```python
from build123d import *

# Parameters (mm, degrees)
SKETCH1_R           = 9
BOSS_EXTRUDE1_DEPTH = 4
SKETCH2_R           = 6
BOSS_EXTRUDE2_DEPTH = 2
SKETCH3_R           = 6.5
BOSS_EXTRUDE3_DEPTH = 54.2
SKETCH4_R           = 5.95
BOSS_EXTRUDE4_DEPTH = 1
SKETCH5_R           = 6.5
BOSS_EXTRUDE5_DEPTH = 4.8
CHAMFER1_SIZE       = 1


with BuildPart() as part:
    # Sketch1 → Boss-Extrude1 (new body)
    with BuildSketch(Plane.XY):
        Circle(SKETCH1_R)
    extrude(amount=BOSS_EXTRUDE1_DEPTH)

    # Sketch2 → Boss-Extrude2 (add)
    with BuildSketch(Plane.XY.offset(4)):
        Circle(SKETCH2_R)
    extrude(amount=BOSS_EXTRUDE2_DEPTH)

    # Sketch3 → Boss-Extrude3 (add)
    with BuildSketch(Plane.XY.offset(6)):
        with Locations(Location((0, 0, 0), (0, 0, 180))):
            Circle(SKETCH3_R)
    extrude(amount=BOSS_EXTRUDE3_DEPTH)

    # Sketch4 → Boss-Extrude4 (add)
    with BuildSketch(Plane.XY.offset(60.2)):
        Circle(SKETCH4_R)
    extrude(amount=BOSS_EXTRUDE4_DEPTH)

    # Sketch5 → Boss-Extrude5 (add)
    with BuildSketch(Plane.XY.offset(61.2)):
        with Locations(Location((0, 0, 0), (0, 0, 180))):
            Circle(SKETCH5_R)
    extrude(amount=BOSS_EXTRUDE5_DEPTH)

    # Chamfer1
    chamfer1_edges = [part.edges().sort_by_distance(p)[0] for p in [
        (-9, 0, 0),
        (6.5, 0, 66),
    ]]
    chamfer(chamfer1_edges, length=CHAMFER1_SIZE)


solid = part.part
```
Geometry: final body of the model. Coordinates: model frame, mm. A direction names the side the tool comes from. Round coordinates to 2 decimals unless told otherwise and drop trailing zeros. Write each loop counter-clockwise with the first axis right and the second up, starting at its lowest first coordinate (ties: lowest second). Pieces come first, ordered by that corner, then holes. Notation, with made-up numbers: (-40, -4) -> (3, -4) arc R13 ccw to (3, 12) -> close; hole circle Ø5 at (54, 3.5). An arc over 180 degrees is marked (long way). Use CSV: the item, a comma, the result in double quotes. Start each with the question number.
Q1. Reachability of faces 4 (the face through (0, 0, 0)), 5 (the face through (5.158, 3.955, 32.721)), 6 (the face through (-6, 0, 5)) from +Z, -Z, +X, -X, +Y, -Y: full face, straight path, thin tool, end or side. Return the list, or none.
Q2. First-contact query: pin 1 Ø6.5 at (x, y) = (-0.5, 2.5) entering from -Z; pin 2 Ø4 at (x, z) = (-0.5, 59) entering from +Y; pin 3 Ø8 at (y, z) = (-5, 13.5) entering from +X; pin 4 Ø10 at (y, z) = (0, 35.5) entering from +X. Flat tips, straight axial feed; report the tip coordinate or a pass-through.
Q3. Line query: L1, parallel to Z at x = 6.25, y = 1.25; L2, parallel to Z at x = 2, y = -7.25; L3, parallel to Y at x = 2.5, z = 53.5. Output: solid intervals per line, ascending.
Q4. Section A-A (x = 0). Return loops of the section in (y, z), plus the area to 3 significant figures.
Q5. Pull-direction query (Z, two-part tool) for faces 1 (the face through (0, 0, 66)), 2 (the face through (-1.172, 8.923, 2.479)), 3 (the face through (-6, 2, 61.2)); classes: pulls with the +Z half, pulls with the -Z half, needs draft (parallel to the pull), parting line crosses it, or undercut.
Q6. Section C-C (z = 59). Return loops of the section in (x, y).
Result sheet:
1,face 4,"-Z, +X, -X, +Y, -Y"
1,face 5,"+Z"
1,face 6,"none"
2,pin 1,"z = 0"
2,pin 2,"y = 6.5"
2,pin 3,"x = 6.42"
2,pin 4,"x = 6.5"
3,L1,"0 to 4, 6 to 60.2, 61.2 to 65.13"
3,L2,"0 to 4"
3,L3,"-6 to 6"
4,outline,"(-9, 1) -> (-8, 0) -> (8, 0) -> (9, 1) -> (9, 4) -> (6, 4) -> (6, 6) -> (6.5, 6) -> (6.5, 60.2) -> (5.95, 60.2) -> (5.95, 61.2) -> (6.5, 61.2) -> (6.5, 65) -> (5.5, 66) -> (-5.5, 66) -> (-6.5, 65) -> (-6.5, 61.2) -> (-5.95, 61.2) -> (-5.95, 60.2) -> (-6.5, 60.2) -> (-6.5, 6) -> (-6, 6) -> (-6, 4) -> (-9, 4) -> close"
4,area,"873 mm²"
5,face 1,"pulls with the +Z half"
5,face 2,"needs draft"
5,face 3,"undercut"
6,outline,"circle Ø13 at (0, 0)"
